from build123d import *

# Parameters (mm, degrees)
G1_4_TAPPED_HOLE1_D                               = 11.8
HOLE_SIZE_BASED_ON_SOCKET_HEAD_CAP_SC_D           = 4.8
HOLE_SIZE_BASED_ON_SOCKET_HEAD_CAP_SC_CBORE_D     = 8
HOLE_SIZE_BASED_ON_SOCKET_HEAD_CAP_SC_CBORE_DEPTH = 4.6
FILLET1_R                                         = 0.2
CHAMFER1_SIZE                                     = 0.2
CHAMFER2_SIZE                                     = 0.5
CUT_EXTRUDE1_DEPTH                                = 35.474628352
SKETCH8_R                                         = 15
CUT_EXTRUDE2_DEPTH                                = 30.145808143


with BuildPart() as part:
    # Sketch2 → Revolve1 (revolve)
    with BuildSketch(Plane.XY, mode=Mode.PRIVATE) as revolve1_sk:
        Polygon((0, 24), (-17.5, 24), (-17.5, 16), (-6.75, 16), (-6.75, 0), (0, 0), align=None)
    revolve(revolve1_sk.sketch.rotate(Axis((0, 0, 0), (0, 1, 0)), 270), axis=Axis((0, 0, 0), (0, 1, 0)))

    # G1/4 Tapped Hole1 (through all)
    with Locations(Plane.ZX.offset(24)):
        with Locations((0, 0)):
            Hole(G1_4_TAPPED_HOLE1_D / 2)

    # Hole Size (% based on) Socket Head Cap Screw Type 1 (through all)
    with Locations(Plane(origin=(-8.485281374, 24, -8.485281374), x_dir=(0, 0, 1), z_dir=(0, 1, 0))):
        with Locations((0, 0), (16.970562748, 16.970562748)):
            CounterBoreHole(HOLE_SIZE_BASED_ON_SOCKET_HEAD_CAP_SC_D / 2, HOLE_SIZE_BASED_ON_SOCKET_HEAD_CAP_SC_CBORE_D / 2, HOLE_SIZE_BASED_ON_SOCKET_HEAD_CAP_SC_CBORE_DEPTH)

    # Fillet1
    fillet1_edges = [part.edges().sort_by_distance(p)[0] for p in [
        (0, 16, 6.75),
    ]]
    fillet(fillet1_edges, radius=FILLET1_R)

    # Chamfer1
    chamfer1_edges = [part.edges().sort_by_distance(p)[0] for p in [
        (0, 0, 6.75),
        (0, 16, 17.5),
        (0, 24, 17.5),
    ]]
    chamfer(chamfer1_edges, length=CHAMFER1_SIZE)

    # Chamfer2
    chamfer2_edges = [part.edges().sort_by_distance(p)[0] for p in [
        (0, 24, 5.9),
        (0, 0, 5.9),
    ]]
    chamfer(chamfer2_edges, length=CHAMFER2_SIZE)

    # Sketch7 → Cut-Extrude1 (cut, through all)
    with BuildSketch(Plane(origin=(0, 24, 0), x_dir=(1, 0, 0), z_dir=(0, 1, 0))):
        with BuildLine():
            Line((2.911166407, -17.053302031), (-17.053302031, 2.911166407))
            ThreePointArc((-17.053302031, 2.911166407), (-12.232947315, -12.232947315), (2.911166407, -17.053302031))
        make_face()
        with BuildLine():
            ThreePointArc((17.3, 0), (11.156317071, 13.222200627), (-2.911166407, 17.053302031))
            Line((-2.911166407, 17.053302031), (17.053302031, -2.911166407))
            ThreePointArc((17.053302031, -2.911166407), (17.238215179, -1.460800272), (17.3, 0))
        make_face()
        with BuildLine():
            Line((-17.053302031, 2.911166407), (-17.226115818, 3.083980194))
            ThreePointArc((-17.226115818, 3.083980194), (-12.374368671, -12.374368671), (3.083980194, -17.226115818))
            Line((3.083980194, -17.226115818), (2.911166407, -17.053302031))
            ThreePointArc((2.911166407, -17.053302031), (-12.232947315, -12.232947315), (-17.053302031, 2.911166407))
        make_face()
        with BuildLine():
            ThreePointArc((17.5, 0), (11.23121424, 13.42050024), (-3.083980194, 17.226115818))
            Line((-3.083980194, 17.226115818), (-2.911166407, 17.053302031))
            ThreePointArc((-2.911166407, 17.053302031), (11.156317071, 13.222200627), (17.3, 0))
            ThreePointArc((17.3, 0), (17.238215179, -1.460800272), (17.053302031, -2.911166407))
            Line((17.053302031, -2.911166407), (17.226115818, -3.083980194))
            ThreePointArc((17.226115818, -3.083980194), (17.431394477, -1.548058977), (17.5, 0))
        make_face()
    extrude(amount=-CUT_EXTRUDE1_DEPTH, mode=Mode.SUBTRACT)

    # Sketch8 → Cut-Extrude2 (cut, through all)
    with BuildSketch(Plane.XZ.offset(-16)):
        Circle(SKETCH8_R)
    extrude(amount=CUT_EXTRUDE2_DEPTH, mode=Mode.SUBTRACT)


solid = part.part
Geometry check sheet. Reference: the model listing, model coordinates, mm. A direction names the side the tool comes from. Give positions to 0.01 mm unless a question says otherwise; leave off trailing zeros. Loops run counter-clockwise (first coordinate to the right, second up) from the corner with the lowest first, then second, coordinate; pieces in that order, holes last. Notation, with made-up numbers: M 60,-12.5 L 118,-12.5 A13 ccw 118,1.5 Z; hole C -26,-14 d2. An arc over 180 degrees is marked long. Answer as a JSON object with one key per item and string values. Group by question number.
Item 1: Sectioned sample at B-B on z = 0. Record the boundary of the cut face in (x, y).
Item 2: Sectioned sample at A-A on x = 0. Record the boundary of the cut face in (y, z).
Item 3: Gauge pin test, flat ends, axial feed: pin 1 (1 mm diameter, centred on x = -8.5, z = 6, fed in from +Y); pin 2 (7.5 mm diameter, centred on x = 8.49, z = 8.49, fed in from +Y); pin 3 (3 mm diameter, centred on y = 18.5, z = 0.5, fed in from -X). Record the tip position at first contact, or that the pin passes through.
Item 4: Sectioned sample at C-C on y = 17. Record the boundary of the cut face in (x, z), plus the area to 3 significant figures.
Item 5: Material ranges on L1, parallel to X at y = 22, z = 3; L2, parallel to X at y = 17, z = -1; L3, parallel to Z at x = 2.5, y = 18.75, recorded low to high.
Item 6: Sectioned sample at D-D on y = 22.25. Record the boundary of the cut face in (x, z), plus the area to 3 significant figures.
Item 7: Access from +Z, -Z, +X, -X, +Y, -Y to the whole of each face (thin tool, end or side, straight path). Record for faces 1 (the cylindrical face through (-12.39, 21.73, -9.35)), 2 (the cylindrical face through (12.27, 19.95, 12.48)).
Item 8: Mould release check, pull along X, two halves, no side actions. Record for faces 3 (the cylindrical face through (10.51, 17.68, 7.2)), 4 (the flat face through (0, 16, 8)), 5 (the flat face through (6.93, 20.06, -7.21)), 6 (the flat face through (-6.93, 20.06, 7.21)): pulls with the +X half, pulls with the -X half, needs draft (parallel to the pull), parting line crosses it, or undercut.
Findings below:
{
 "1": {"outline": "M -14.14,16 L -5.9,16 L -5.9,23.5 L -6.4,24 L -14.14,24 Z; M 5.9,16 L 14.14,16 L 14.14,24 L 6.4,24 L 5.9,23.5 Z"},
 "2": {"outline": "M 16,-14.14 L 24,-14.14 L 24,-6.4 L 23.5,-5.9 L 16,-5.9 Z; M 16,5.9 L 23.5,5.9 L 24,6.4 L 24,14.14 L 16,14.14 Z"},
 "3": {"pin 1": "y = 24", "pin 2": "y = 19.4", "pin 3": "x = -15.14"},
 "4": {"outline": "M -17.23,-3.08 A17.5 ccw -3.08,-17.23 L 17.23,3.08 A17.5 ccw 3.08,17.23 Z; hole C -8.49,-8.49 d4.8; hole C 0,0 d11.8; hole C 8.49,8.49 d4.8", "area": "514 mm2"},
 "5": {"L1": "-11.14 to -5.08, 5.08 to 17.14", "L2": "-15.14 to -5.81, 5.81 to 13.14", "L3": "-11.64 to -5.34, 5.34 to 16.64"},
 "6": {"outline": "M -17.23,-3.08 A17.5 ccw -3.08,-17.23 L 17.23,3.08 A17.5 ccw 3.08,17.23 Z; hole C -8.49,-8.49 d8; hole C 0,0 d11.8; hole C 8.49,8.49 d8", "area": "450 mm2"},
 "7": {"face 1": "+Y", "face 2": "+Z, +X, +Y, -Y"},
 "8": {"face 3": "undercut", "face 4": "needs draft", "face 5": "pulls with the +X half", "face 6": "pulls with the -X half"}
}
